The model under review builds one solid part; all positions refer to its coordinate system, in mm. Face numbers are marked on the shaded views. A direction names the side the tool comes from. Round coordinates to 2 decimals unless told otherwise and drop trailing zeros. Write each loop counter-clockwise with the first axis right and the second up, starting at its lowest first coordinate (ties: lowest second). Pieces come first, ordered by that corner, then holes. Notation, with made-up numbers: M -23,10.25 L 2,10.25 A23 ccw 2,32.25 Z; hole C -24.5,-3 d7. An arc over 180 degrees is marked long. One line per item, written item: value. Start each with the question number.
1) Take a section at B-B, the plane y = -4.25. Write out the cut boundary in (x, z).
2) Mouldability with a two-part tool opening along Y and no side actions: class the marked faces 1 and 2 as +Y half, -Y half, draft (parallel to the pull), parting line (faces both ways), or undercut.
3) For P1, Ø5, axis at y = 2.5, z = 10.5, coming from the +X side; P2, Ø1, axis at x = 4, y = -1.5, coming from the +Z side; P3, Ø8, axis at y = 5.5, z = 35, coming from the +X side, all flat-tipped, find the tip position at first contact; note any pin that passes through.
4) Take a section at A-A, the plane x = 0. Write out the cut boundary in (y, z), and give its area (3 significant figures).
5) Wall thickness on probe 1 along Z at (x, y) = (0.75, -6); probe 2 along X at (y, z) = (4, 4.5); probe 3 along X at (y, z) = (3.75, 21): over which ranges is each line inside the solid? List them lowest first.
6) Take a section at C-C, the plane z = 10. Write out the cut boundary in (x, y).
7) Tool access review of the marked faces 3 and 4: name each direction out of +Z, -Z, +X, -X, +Y, -Y from which nothing blocks a thin tool from reaching the whole face with its end or side.
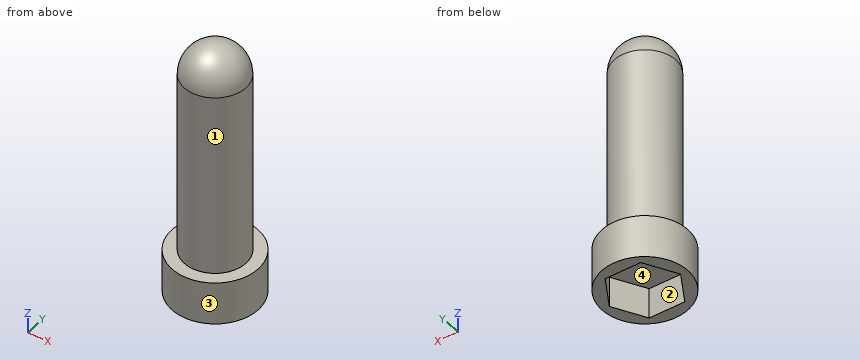
from build123d import *

# Parameters (mm, degrees)
HEAD_PROFILE_SKETCH_R       = 7
HEAD_14X10_DEPTH            = 7
SHANK_PROFILE_SKETCH_R      = 5
SHANK_10X35_DEPTH           = 35
DOMED_END_R5_R              = 5
HEX_SOCKET_CUT_5_DEEP_DEPTH = 5


with BuildPart() as part:
    # Head Profile Sketch → Head Ø14x10 (new body)
    with BuildSketch(Plane.XY):
        Circle(HEAD_PROFILE_SKETCH_R)
    extrude(amount=HEAD_14X10_DEPTH)

    # Shank Profile Sketch → Shank Ø10x35 (add)
    with BuildSketch(Plane.XY.offset(7)):
        Circle(SHANK_PROFILE_SKETCH_R)
    extrude(amount=SHANK_10X35_DEPTH)

    # Domed End R5
    domed_end_r5_edges = [part.edges().sort_by_distance(p)[0] for p in [
        (-5, 0, 42),
    ]]
    fillet(domed_end_r5_edges, radius=DOMED_END_R5_R)

    # Hex Socket Sketch → Hex Socket Cut 5 Deep (cut)
    with BuildSketch(Plane(origin=(0, 0, 0), x_dir=(-1, 0, 0), z_dir=(0, 0, -1))):
        Polygon((5.773502692, 0), (2.886751346, 5), (-2.886751346, 5), (-5.773502692, 0), (-2.886751346, -5), (2.886751346, -5), align=None)
    extrude(amount=-HEX_SOCKET_CUT_5_DEEP_DEPTH, mode=Mode.SUBTRACT)


solid = part.part
Checked values:
1. outline: M -5.56,0 L -3.32,0 L -3.32,5 L 3.32,5 L 3.32,0 L 5.56,0 L 5.56,7 L 2.63,7 L 2.63,37 A2.63 ccw -2.63,37 L -2.63,7 L -5.56,7 Z
2. face 1: parting line
2. face 2: undercut
3. P1: stops at x = 5
3. P2: stops at z = 40.28
3. P3: stops at x = 4.77
4. outline: M -7,0 L -5,0 L -5,5 L 5,5 L 5,0 L 7,0 L 7,7 L 5,7 L 5,37 A5 ccw -5,37 L -5,7 L -7,7 Z
4. area: 387 mm2
5. probe 1: z = 0 to 7
5. probe 2: x = -5.74 to -3.46, 3.46 to 5.74
5. probe 3: x = -3.31 to 3.31
6. outline: C 0,0 d10
7. face 3: +Z, -Z
7. face 4: -Z
